Geometry check sheet. Reference: the model listing, model coordinates, mm. A direction names the side the tool comes from. Round coordinates to 2 decimals unless told otherwise and drop trailing zeros. Order: outer loops, then holes, each group sorted by start corner. A loop starts at its lowest first (then second) coordinate and runs counter-clockwise, first axis right, second up. Notation, with made-up numbers: (-21, -16.5) -> (-1, -16.5) arc R9 cw to (-1, -8.5) -> close; hole circle Ø10 at (-27.5, 1). An arc over 180 degrees is marked (long way). Use a Markdown table: item, result. Add a question column.
Item 1: Sectioned sample at D-D, the plane z = 23. Record the cut outline in (x, y), and give its area (3 significant figures).
Item 2: Set-up check for faces 1 (the cylindrical face through (11.923, 3.755, 59.972)), 2 (the flat face through (0, 0, 92)): record each of +Z, -Z, +X, -X, +Y, -Y from which the full face is reachable in a straight line by a thin tool's end or side.
Item 3: Sectioned sample at A-A, the plane y = 0. Record the cut outline in (x, z), and give its area (3 significant figures).
Item 4: Material ranges on probe 1 along Z at (x, y) = (0, 1.5); probe 2 along X at (y, z) = (-5, 77); probe 3 along X at (y, z) = (1.5, 77), recorded low to high. Write a range as [from, to].
Item 5: Sectioned sample at B-B, the plane x = 0. Record the cut outline in (y, z).
Item 6: Gauge pin test, flat ends, axial feed: pin 1 Ø1 at (y, z) = (5, 17) entering from -X; pin 2 Ø12 at (y, z) = (-6, 31.5) entering from +X; pin 3 Ø12 at (y, z) = (-10, 18) entering from +X. Record the tip position at first contact, or that the pin passes through.
Item 7: Mould release check, pull along X, two halves, no side actions. Record for faces 3 (the flat face through (0, 0, 0)), 4 (the cylindrical face through (6.437, -12.376, 76.297)), 5 (the cylindrical face through (-1.8, 0.2, 74.6)): pulls with the +X half, pulls with the -X half, needs draft (parallel to the pull), parting line crosses it, or undercut.
Item 8: Sectioned sample at C-C, the plane z = 77. Record the cut outline in (x, y).
from build123d import *

# Parameters (mm, degrees)
SKETCH_1_R          = 10
EXTRUDE_1_DEPTH     = 58
SKETCH_2_R          = 12.5
EXTRUDE_2_DEPTH     = 4
SKETCH_3_R          = 13.95
EXTRUDE_3_DEPTH     = 30
CHAMFER_1_SIZE      = 1
FILLET_1_R          = 0.5
SKETCH_4_R          = 3
CUT_EXTRUDE_1_DEPTH = 15


with BuildPart() as part:
    # 草图1 → 凸台-拉伸1 (new body)
    with BuildSketch(Plane.XY):
        with Locations(Location((0, 0, 0), (0, 0, 180))):
            Circle(SKETCH_1_R)
    extrude(amount=EXTRUDE_1_DEPTH)

    # 草图2 → 凸台-拉伸2 (add)
    with BuildSketch(Plane.XY.offset(58)):
        Circle(SKETCH_2_R)
    extrude(amount=EXTRUDE_2_DEPTH)

    # 草图3 → 凸台-拉伸3 (add)
    with BuildSketch(Plane.XY.offset(62)):
        Circle(SKETCH_3_R)
    extrude(amount=EXTRUDE_3_DEPTH)

    # 倒角1
    chamfer_1_edges = [part.edges().sort_by_distance(p)[0] for p in [
        (-13.95, 0, 92),
        (10, 0, 0),
    ]]
    chamfer(chamfer_1_edges, length=CHAMFER_1_SIZE)

    # 圆角1
    fillet_1_edges = [part.edges().sort_by_distance(p)[0] for p in [
        (10, 0, 58),
    ]]
    fillet(fillet_1_edges, radius=FILLET_1_R)

    # 草图4 → 切除-拉伸1 (cut, symmetric)
    with BuildSketch(Plane(origin=(0, 0, 0), x_dir=(1, 0, 0), z_dir=(0, 1, 0))):
        with Locations(Location((0, -77, 0), (0, 0, 270))):
            Circle(SKETCH_4_R)
    extrude(amount=CUT_EXTRUDE_1_DEPTH, both=True, mode=Mode.SUBTRACT)


solid = part.part
Found:
| question | item | result |
|---|---|---|
| 1 | outline | circle Ø20 at (0, 0) |
| 1 | area | 314 mm2 |
| 2 | face 1 | -Z |
| 2 | face 2 | +Z, +X, -X, +Y, -Y |
| 3 | outline | (-13.95, 62) -> (-12.5, 62) -> (-12.5, 58) -> (-10.5, 58) arc R0.5 cw to (-10, 57.5) -> (-10, 1) -> (-9, 0) -> (9, 0) -> (10, 1) -> (10, 57.5) arc R0.5 cw to (10.5, 58) -> (12.5, 58) -> (12.5, 62) -> (13.95, 62) -> (13.95, 91) -> (12.95, 92) -> (-12.95, 92) -> (-13.95, 91) -> close; hole circle Ø6 at (0, 77) |
| 3 | area | 2,070 mm2 |
| 4 | probe 1 | z = [0, 74], [80, 92] |
| 4 | probe 2 | x = [-13.02, -3], [3, 13.02] |
| 4 | probe 3 | x = [-13.87, -3], [3, 13.87] |
| 5 | outline | (-13.95, 62) -> (-12.5, 62) -> (-12.5, 58) -> (-10.5, 58) arc R0.5 cw to (-10, 57.5) -> (-10, 1) -> (-9, 0) -> (9, 0) -> (10, 1) -> (10, 57.5) arc R0.5 cw to (10.5, 58) -> (12.5, 58) -> (12.5, 62) -> (13.95, 62) -> (13.95, 74) -> (-13.95, 74) -> close; (-13.95, 80) -> (13.95, 80) -> (13.95, 91) -> (12.95, 92) -> (-12.95, 92) -> (-13.95, 91) -> close |
| 6 | pin 1 | stops at x = -8.93 |
| 6 | pin 2 | stops at x = 10 |
| 6 | pin 3 | stops at x = 9.17 |
| 7 | face 3 | needs draft |
| 7 | face 4 | parting line crosses it |
| 7 | face 5 | undercut |
| 8 | outline | (-3, -13.62) -> (-3, 13.62) arc R13.95 ccw to start; (3, -13.62) arc R13.95 ccw to (3, 13.62) -> close |
